The model under review builds one solid part; all positions refer to its coordinate system, in mm. Face numbers are marked on the shaded views. A direction names the side the tool comes from. Coordinates: 2 decimals unless noted, no trailing zeros. Order: outer loops, then holes, each group sorted by start corner. A loop starts at its lowest first (then second) coordinate and runs counter-clockwise, first axis right, second up.
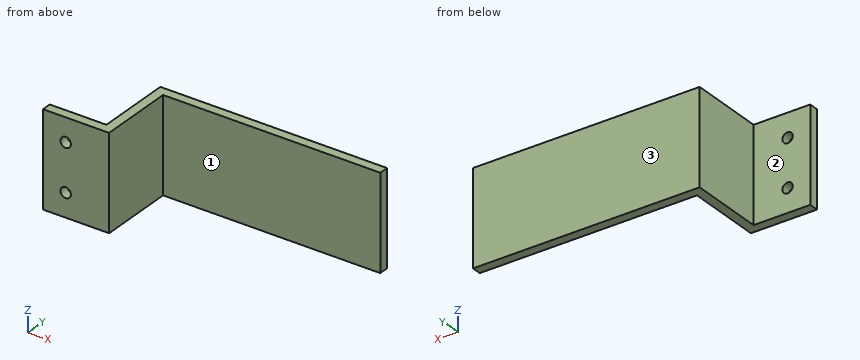
```python
from build123d import *

# Parameters (mm, degrees)
EXTRUDE_1_DEPTH     = 50
SKETCH_2_R          = 2.75
CUT_EXTRUDE_1_DEPTH = 10


with BuildPart() as part:
    # 草图1 → 拉伸-薄壁1 (new body)
    with BuildSketch(Plane.XY):
        Polygon((0, 0), (30, 0), (30, 40), (150, 40), (150, 35), (35, 35), (35, -5), (0, -5), align=None)
    extrude(amount=EXTRUDE_1_DEPTH)

    # 草图2 → 切除-拉伸1 (cut)
    with BuildSketch(Plane(origin=(0, 0, 0), x_dir=(1, 0, 0), z_dir=(0, 1, 0))):
        with Locations(Location((12, -12.5, 0), (0, 0, 270))):
            Circle(SKETCH_2_R)
        with Locations(Location((12, -37.5, 0), (0, 0, 270))):
            Circle(SKETCH_2_R)
    extrude(amount=-CUT_EXTRUDE_1_DEPTH, mode=Mode.SUBTRACT)


solid = part.part
```
(1) We need section B-B, the plane x = 12. Write out the cut boundary in (y, z).
A:
outline: (-5, 0) - (0, 0) - (0, 9.75) - (-5, 9.75) - close; (-5, 15.25) - (0, 15.25) - (0, 34.75) - (-5, 34.75) - close; (-5, 40.25) - (0, 40.25) - (0, 50) - (-5, 50) - close
(2) We need section D-D, the plane y = 21.5. Write out the cut boundary in (x, z).
A:
outline: (30, 0) - (35, 0) - (35, 50) - (30, 50) - close
(3) Wall thickness on probe 1 along X at (y, z) = (-1.3, 12.5); probe 2 along X at (y, z) = (9, 46); probe 3 along Y at (x, z) = (28, 43): over which ranges is each line inside the solid? List them lowest first.
A:
probe 1: x = 0 to 9.25, 14.75 to 35
probe 2: x = 30 to 35
probe 3: y = -5 to 0
(4) We need section C-C, the plane z = 47. Write out the cut boundary in (x, y), and give its area (3 significant figures).
A:
outline: (0, -5) - (35, -5) - (35, 35) - (150, 35) - (150, 40) - (30, 40) - (30, 0) - (0, 0) - close
area: 950 mm2
(5) Machinability: for the marked faces 1, 2 and 3, which of the approach directions +Z, -Z, +X, -X, +Y, -Y give a long, thin tool a straight path to every point of the face, cutting with its end or side? Answer none if there is none.
A:
face 1: +Z, -Z, +X, -Y
face 2: +Z, -Z, -X, +Y
face 3: +Z, -Z, +X, -X, +Y
(6) For pin 1 Ø8 at (y, z) = (28, 15.5) entering from -X; pin 2 Ø5 at (x, z) = (39.5, 45) entering from -Y; pin 3 Ø4.5 at (x, z) = (12, 12.5) entering from -Y; pin 4 Ø9 at (x, z) = (12, 34) entering from +Y, all flat-tipped, find the tip position at first contact; note any pin that passes through.
A:
pin 1: stops at x = 30
pin 2: stops at y = 35
pin 3: passes through
pin 4: stops at y = 0
(7) We need section A-A, the plane z = 37.5. Write out the cut boundary in (x, y), and give its area (4 significant figures).
A:
outline: (0, -5) - (9.25, -5) - (9.25, 0) - (0, 0) - close; (14.75, -5) - (35, -5) - (35, 35) - (150, 35) - (150, 40) - (30, 40) - (30, 0) - (14.75, 0) - close
area: 922.5 mm2
